The drawing under review shows one solid part. Ordinate dimensions are in mm from its lowest x, y, z. A direction names the side the tool comes from. Coordinates: 2 decimals unless noted, no trailing zeros. Loops run counter-clockwise (first coordinate to the right, second up) from the corner with the lowest first, then second, coordinate; pieces in that order, holes last. Notation, with made-up numbers: M 8,83.5 L 33,83.5 A35 cw 33,122.5 Z; hole C 78.25,89 d11. An arc over 180 degrees is marked long. Answer as a JSON object with one key per item and string values. Group by question number.
1. Machinability: for the marked faces 4, 5, 6 and 7, which of the approach directions +Z, -Z, +X, -X, +Y, -Y give a long, thin tool a straight path to every point of the face, cutting with its end or side? Answer none if there is none.
2. Consider section A-A (y = 7.5). State the section outline as (x, z) points, then the cut area to 3 significant figures.
3. Consider section D-D (y = 18.25). State the section outline as (x, z) points, then the cut area to 3 significant figures.
4. Consider section C-C (x = 16). State the section outline as (y, z) points.
5. Insertion check: pin 1 (1 mm diameter, centred on y = 14.5, z = 2.5, fed in from -X); pin 2 (1.5 mm diameter, centred on x = 6.5, z = 4.5, fed in from +Y); pin 3 (1.8 mm diameter, centred on x = 15, y = 8.5, fed in from +Z); pin 4 (3 mm diameter, centred on y = 2.5, z = 1.5, fed in from +X). Each pin has a flat end and moves straight along its axis. Give the tip position at first contact, or say it passes through.
6. To check wall thickness, follow probe 1 along X at (y, z) = (9.25, 8.5); probe 2 along X at (y, z) = (17.5, 6); probe 3 along Y at (x, z) = (13.5, 7.25). State the ranges of each line that lie inside material, in increasing order.
7. Draft analysis for pull direction X (two halves, no side actions). For the marked faces 1, 2 and 3, state which applies: +X half, -X half, draft (parallel to the pull), parting line (faces both ways), or undercut.
8. Consider section B-B (z = 5). State the section outline as (x, y) points.
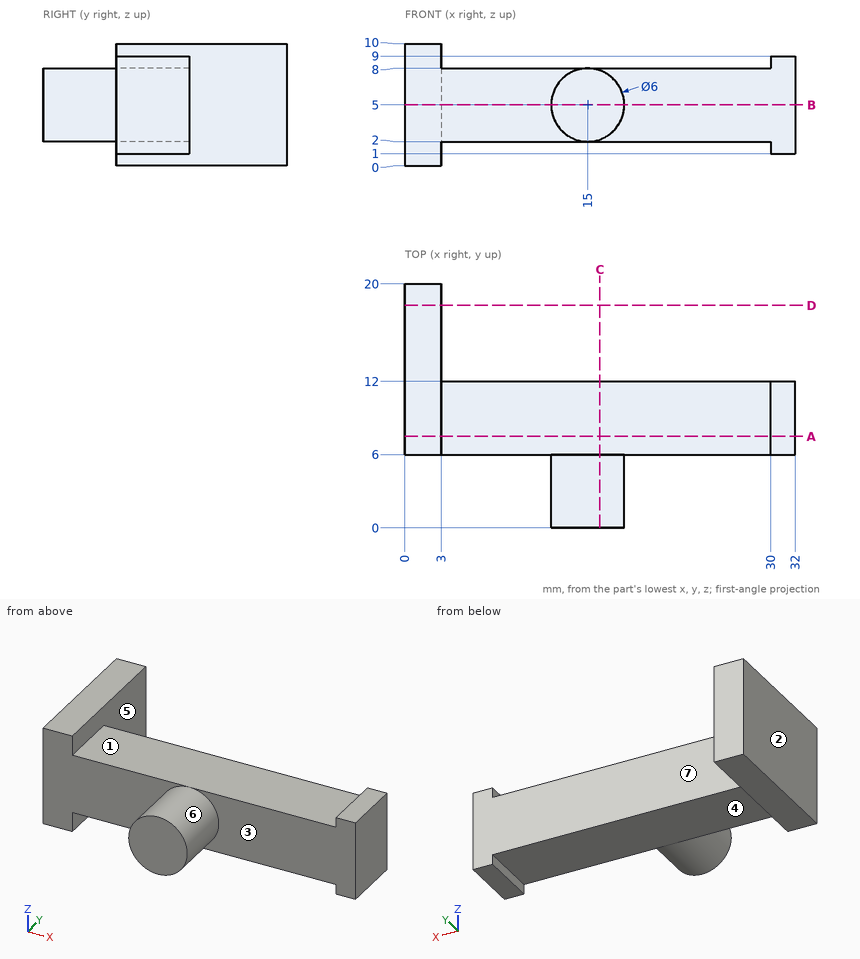
Findings below:
{
 "1": {"face 4": "-Z, +Y, -Y", "face 5": "+Y", "face 6": "-Y", "face 7": "+Z, -Z, +X, +Y"},
 "2": {"outline": "M 0,0 L 3,0 L 3,2 L 30,2 L 30,1 L 32,1 L 32,9 L 30,9 L 30,8 L 3,8 L 3,10 L 0,10 Z", "area": "208 mm^2"},
 "3": {"outline": "M 0,0 L 3,0 L 3,10 L 0,10 Z", "area": "30.0 mm^2"},
 "4": {"outline": "M 0,2.17 L 6,2.17 L 6,2 L 12,2 L 12,8 L 6,8 L 6,7.83 L 0,7.83 Z"},
 "5": {"pin 1": "stops at x = 0", "pin 2": "stops at y = 12", "pin 3": "stops at z = 8", "pin 4": "stops at x = 17.24"},
 "6": {"probe 1": "x = 0 to 3, 30 to 32", "probe 2": "x = 0 to 3", "probe 3": "y = 0 to 12"},
 "7": {"face 1": "undercut", "face 2": "-X half", "face 3": "draft"},
 "8": {"outline": "M 0,6 L 12,6 L 12,0 L 18,0 L 18,6 L 32,6 L 32,12 L 3,12 L 3,20 L 0,20 Z"}
}
